Source: CAD feature listing. Evaluate the final solid. Frame: model axes, mm. A direction names the side the tool comes from. Round coordinates to 2 decimals unless told otherwise and drop trailing zeros. Use a Markdown table: item, result. Add a question column.
```python
from build123d import *

# Parameters (mm, degrees)
SKETCH_1_W                     = 670
SKETCH_1_H                     = 140
EXTRUDE_1_DEPTH                = 16
HOLE_WIZARD_M8_1_D             = 6.8
HOLE_WIZARD_M6_1_D             = 5
HOLE_WIZARD_M8_1_2_D           = 9
HOLE_WIZARD_M8_1_2_CBORE_D     = 15
HOLE_WIZARD_M8_1_2_CBORE_DEPTH = 8.6
SKETCH_16_W                    = 670
SKETCH_16_H                    = 20
CUT_EXTRUDE_1_DEPTH            = 343.609106709
SKETCH_19_W                    = 10
SKETCH_19_H                    = 120
CUT_EXTRUDE_2_DEPTH            = 343.609106709
CHAMFER_1_SIZE                 = 3
HOLE_WIZARD_M6_2_D             = 5
HOLE_WIZARD_M4_1_D             = 3.3


with BuildPart() as part:
    # 草图1 → 凸台-拉伸1 (new body)
    with BuildSketch(Plane.XY):
        Rectangle(SKETCH_1_W, SKETCH_1_H)
    extrude(amount=EXTRUDE_1_DEPTH)

    # Hole Wizard M8 _1 (through all)
    with Locations(Plane.XY.offset(16)):
        with Locations((-305, 57.5), (-305, 27.5), (305, 27.5), (305, 57.5)):
            Hole(HOLE_WIZARD_M8_1_D / 2)

    # M6 螺纹孔1 (through all)
    with Locations(Plane.XY.offset(16)):
        with Locations((-270, 42.5), (-210, 42.5), (-150, 42.5), (-90, 42.5), (-30, 42.5), (30, 42.5), (90, 42.5), (150, 42.5), (210, 42.5), (270, 42.5)):
            Hole(HOLE_WIZARD_M6_1_D / 2)

    # Hole Wizard M8 _1 2 (through all)
    with Locations(Plane.XY.offset(16)):
        with Locations((290, -30), (145, -30), (0, -30), (-145, -30), (-290, -30), (-435, -30)):
            CounterBoreHole(HOLE_WIZARD_M8_1_2_D / 2, HOLE_WIZARD_M8_1_2_CBORE_D / 2, HOLE_WIZARD_M8_1_2_CBORE_DEPTH)

    # 草图16 → 切除-拉伸1 (cut, through all)
    with BuildSketch(Plane.XY.offset(16)):
        with Locations((0, -60)):
            Rectangle(SKETCH_16_W, SKETCH_16_H)
    extrude(amount=-CUT_EXTRUDE_1_DEPTH, mode=Mode.SUBTRACT)

    # 草图19 → 切除-拉伸2 (cut, through all)
    with BuildSketch(Plane.XY.offset(16)):
        with Locations((-330, 10)):
            Rectangle(SKETCH_19_W, SKETCH_19_H)
    cut_extrude_2 = extrude(amount=-CUT_EXTRUDE_2_DEPTH, mode=Mode.SUBTRACT)

    # 镜向1: 切除-拉伸2 across plane
    add(cut_extrude_2.mirror(Plane(origin=(0, 0, 0), x_dir=(0, 0, 1), z_dir=(1, 0, 0))), mode=Mode.SUBTRACT)

    # 倒角1
    chamfer_1_edges = [part.edges().sort_by_distance(p)[0] for p in [
        (-325, 70, 8),
        (-325, -50, 8),
        (325, -50, 8),
        (325, 70, 8),
    ]]
    chamfer(chamfer_1_edges, length=CHAMFER_1_SIZE)

    # M6 螺纹孔2 (through all)
    with Locations(Plane.XY.offset(16)):
        with Locations((-310, -11), (-310, -36), (310, -11), (310, -36)):
            Hole(HOLE_WIZARD_M6_2_D / 2)

    # M4 螺纹孔1 (through all)
    with Locations(Plane.XY.offset(16)):
        with Locations((277.5, -36.25), (-277.5, -36.25)):
            Hole(HOLE_WIZARD_M4_1_D / 2)


solid = part.part
```
1) First-contact query: pin 1 Ø10 at (x, y) = (-77.5, -31.5) entering from -Z. Flat tip, straight axial feed; report the tip coordinate or a pass-through.
2) Reachability of faces 4 (the flat face through (-5, -50, 8)), 5 (the cylindrical face through (-1.63, -37.32, 11.76)) from +Z, -Z, +X, -X, +Y, -Y: full face, straight path, thin tool, end or side. Return the list, or none.
3) Line query: probe 1 along Y at (x, z) = (139, 15.25); probe 2 along Y at (x, z) = (210, 5.75); probe 3 along X at (y, z) = (56, 7). Output: solid intervals per line, ascending. Write a range as from..to.
4) Draft query along Y for faces 1 (the flat face through (325, 9, 8)), 2 (the flat face through (-285, -30, 7.4)), 3 (the flat face through (-5, 70, 8)). Return one class per face: pulls with the +Y half, pulls with the -Y half, needs draft (parallel to the pull), parting line crosses it, or undercut.
5) Section A-A on z = 13. Count the separate pieces of the cut face and the enclosed holes in it, then the cut area to 3 significant figures.
Conclusion:
| question | item | result |
|---|---|---|
| 1 | pin 1 | stops at z = 0 |
| 2 | face 4 | +Z, -Z, +X, -X, -Y |
| 2 | face 5 | +Z |
| 3 | probe 1 | y = -50..-34.5, -25.5..70 |
| 3 | probe 2 | y = -50..40, 45..70 |
| 3 | probe 3 | x = -325..-308.05, -301.95..301.95, 308.05..325 |
| 4 | face 1 | needs draft |
| 4 | face 2 | undercut |
| 4 | face 3 | pulls with the +Y half |
| 5 | separate pieces | 1 |
| 5 | enclosed holes | 25 |
| 5 | area | 76,700 mm^2 |
